Design review of the part built by this model. Coordinates are the model's own, in mm. Face numbers are marked on the shaded views. A direction names the side the tool comes from. Give positions to 0.01 mm unless a question says otherwise; leave off trailing zeros. Write each loop counter-clockwise with the first axis right and the second up, starting at its lowest first coordinate (ties: lowest second). Pieces come first, ordered by that corner, then holes.
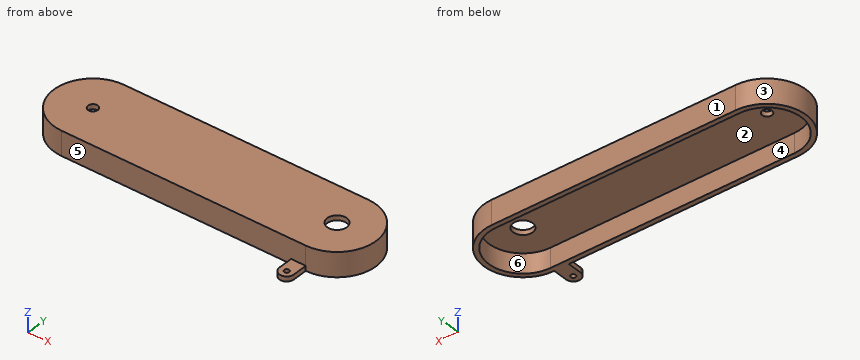
```python
from build123d import *

# Parameters (mm, degrees)
SKETCH_1_R      = 20
SKETCH_1_R_2    = 10
EXTRUDE_1_DEPTH = 10
EXTRUDE_START   = 40
EXTRUDE_2_DEPTH = 40
SKETCH_4_R      = 5
EXTRUDE_3_DEPTH = 10


with BuildPart() as part:
    # 草图1 → 凸台-拉伸1 (new body)
    with BuildSketch(Plane.XY):
        with BuildLine():
            Line((0, 80), (-500, 80))
            ThreePointArc((-500, 80), (-580, 0), (-500, -80))
            Line((-500, -80), (0, -80))
            ThreePointArc((0, -80), (80, 0), (0, 80))
        make_face()
        Circle(SKETCH_1_R, mode=Mode.SUBTRACT)
        with Locations((-500, 0)):
            Circle(SKETCH_1_R_2, mode=Mode.SUBTRACT)
    extrude(amount=EXTRUDE_1_DEPTH)

    # 草图2 → 凸台-拉伸2 (add)
    with BuildSketch(Plane(origin=(0, 0, 0), x_dir=(-1, 0, 0), z_dir=(0, 0, -1)).offset(EXTRUDE_START)):
        with BuildLine():
            Line((0, -80), (500, -80))
            ThreePointArc((500, -80), (580, 0), (500, 80))
            Line((500, 80), (0, 80))
            ThreePointArc((0, 80), (-80, 0), (0, -80))
        make_face()
        with BuildLine():
            Line((0, -70), (500, -70))
            ThreePointArc((500, -70), (570, 0), (500, 70))
            Line((500, 70), (0, 70))
            ThreePointArc((0, 70), (-70, 0), (0, -70))
        make_face(mode=Mode.SUBTRACT)
    extrude(amount=-EXTRUDE_2_DEPTH)

    # 草图4 → 凸台-拉伸3 (add)
    with BuildSketch(Plane(origin=(0, 0, -40), x_dir=(-1, 0, 0), z_dir=(0, 0, -1))):
        with BuildLine():
            Line((30, -110), (30, -80))
            Line((30, -80), (0, -80))
            Line((0, -80), (0, -110))
            ThreePointArc((0, -110), (15, -125.000001141), (30, -110))
        make_face()
        with Locations(Location((15, -110.000001141, 0), (0, 0, 180))):
            Circle(SKETCH_4_R, mode=Mode.SUBTRACT)
    extrude(amount=-EXTRUDE_3_DEPTH)


solid = part.part
```
(1) To check wall thickness, follow L1, parallel to Y at x = -15, z = -36; L2, parallel to Y at x = -500, z = 8; L3, parallel to Y at x = -225, z = -22.5. State the ranges of each line that lie inside material, in increasing order.
Resolved:
L1: y = -125 to -115, -105 to -70, 70 to 80
L2: y = -80 to -10, 10 to 80
L3: y = -80 to -70, 70 to 80
(2) Clearance check with flat-ended pins moving along their axes: P1, Ø2, axis at x = -97.5, y = -28, coming from the -Z side; P2, Ø4, axis at y = -27.5, z = -11, coming from the -X side; P3, Ø1, axis at y = 20, z = 4, coming from the +X side. State where each tip first meets the part, or that it passes through.
Resolved:
P1: stops at z = 0
P2: stops at x = -575.83
P3: stops at x = 77.59
(3) Consider section D-D, the plane y = -90. Give the boundary of the cut face in (x, z), then the cut area to 3 significant figures.
Resolved:
outline: (-30, -40) - (0, -40) - (0, -30) - (-30, -30) - close
area: 300 mm2
(4) Consider section C-C, the plane y = -46.5. Give the boundary of the cut face in (x, z), then the cut area to 3 significant figures.
Resolved:
outline: (-565.1, -40) - (-552.32, -40) - (-552.32, 0) - (52.32, 0) - (52.32, -40) - (65.1, -40) - (65.1, 10) - (-565.1, 10) - close
area: 7,320 mm2
(5) Tool access review of the marked faces 1 and 2: name each direction out of +Z, -Z, +X, -X, +Y, -Y from which nothing blocks a thin tool from reaching the whole face with its end or side.
Resolved:
face 1: +Z, -Z, +X, -X, +Y
face 2: -Z
(6) Mouldability with a two-part tool opening along X and no side actions: class the marked faces 3, 4, 5 and 6 as pulls with the +X half, pulls with the -X half, needs draft (parallel to the pull), parting line crosses it, or undercut.
Resolved:
face 3: pulls with the -X half
face 4: undercut
face 5: needs draft
face 6: undercut
(7) Consider section B-B, the plane x = -226. Give the boundary of the cut face in (y, z).
Resolved:
outline: (-80, -40) - (-70, -40) - (-70, 0) - (70, 0) - (70, -40) - (80, -40) - (80, 10) - (-80, 10) - close
(8) Consider section A-A, the plane z = -23.5. Give the boundary of the cut face in (x, y).
Resolved:
outline: (-500, -80) - (0, -80) arc R80 ccw to (0, 80) - (-500, 80) arc R80 ccw to start; hole (-500, -70) - (0, -70) arc R70 ccw to (0, 70) - (-500, 70) arc R70 ccw to start
